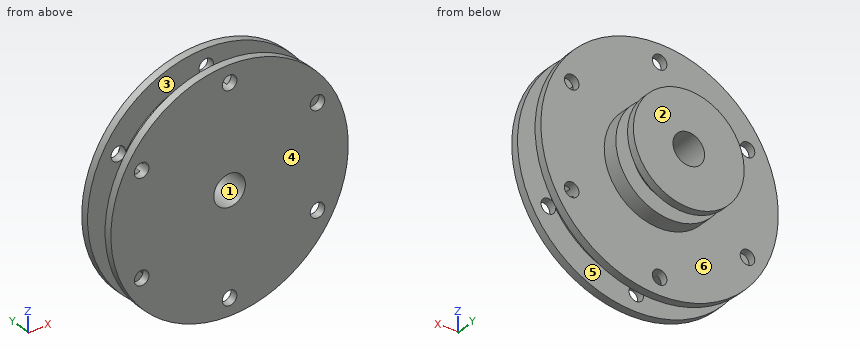
```python
from build123d import *

# Parameters (mm, degrees)
SKETCH1_R               = 15
BOSS_EXTRUDE1_DEPTH     = 5
SKETCH2_W               = 3
SKETCH2_H               = 3
SKETCH3_R               = 7
BOSS_EXTRUDE2_DEPTH     = 5
SKETCH4_W               = 2
SKETCH4_H               = 2
SKETCH5_R               = 2
CUT_EXTRUDE1_DEPTH      = 24.452078799
CUT_EXTRUDE2_DEPTH      = 22.794494718
CUT_EXTRUDE2_DEPTH_BACK = 22.794494718
SKETCH6_R               = 0.920579976


with BuildPart() as part:
    # Sketch1 → Boss-Extrude1 (new body)
    with BuildSketch(Plane(origin=(0, 0, 0), x_dir=(1, 0, 0), z_dir=(0, 1, 0))):
        with Locations(Location((0, 0, 0), (0, 0, 270))):
            Circle(SKETCH1_R)
    extrude(amount=BOSS_EXTRUDE1_DEPTH)

    # Sketch2 → Cut-Revolve1 (revolve, cut)
    with BuildSketch(Plane.XY, mode=Mode.PRIVATE) as cut_revolve1_sk:
        with Locations((13.5, 2.5)):
            Rectangle(SKETCH2_W, SKETCH2_H)
    revolve(cut_revolve1_sk.sketch.rotate(Axis((0, 0, 0), (0, 1, 0)), 90), axis=Axis((0, 0, 0), (0, 1, 0)), mode=Mode.SUBTRACT)

    # Sketch3 → Boss-Extrude2 (add)
    with BuildSketch(Plane(origin=(0, 5, 0), x_dir=(1, 0, 0), z_dir=(0, 1, 0))):
        with Locations(Location((0, 0, 0), (0, 0, 270))):
            Circle(SKETCH3_R)
    extrude(amount=BOSS_EXTRUDE2_DEPTH)

    # Sketch4 → Cut-Revolve2 (revolve, cut)
    with BuildSketch(Plane.XY, mode=Mode.PRIVATE) as cut_revolve2_sk:
        with Locations((6, 8)):
            Rectangle(SKETCH4_W, SKETCH4_H)
    revolve(cut_revolve2_sk.sketch.rotate(Axis((0, 0, 0), (0, 1, 0)), 90), axis=Axis((0, 0, 0), (0, 1, 0)), mode=Mode.SUBTRACT)

    # Sketch5 → Cut-Extrude1 (cut, through all)
    with BuildSketch(Plane(origin=(0, 10, 0), x_dir=(1, 0, 0), z_dir=(0, 1, 0))):
        with Locations(Location((0, 0, 0), (0, 0, 270))):
            Circle(SKETCH5_R)
    extrude(amount=-CUT_EXTRUDE1_DEPTH, mode=Mode.SUBTRACT)

    # Sketch6 → Cut-Extrude2 (cut, two sides: drawn at the far end of the back side and taken through both)
    with BuildSketch(Plane(origin=(0, 5, 0), x_dir=(1, 0, 0), z_dir=(0, 1, 0)).offset(-CUT_EXTRUDE2_DEPTH_BACK)):
        with Locations(Location((0, 12.829886063, 0), (0, 0, 270))):
            Circle(SKETCH6_R)
        with Locations(Location((11.111007258, 6.414943031, 0), (0, 0, 270))):
            Circle(SKETCH6_R)
        with Locations(Location((11.111007258, -6.414943031, 0), (0, 0, 270))):
            Circle(SKETCH6_R)
        with Locations(Location((0, -12.829886063, 0), (0, 0, 270))):
            Circle(SKETCH6_R)
        with Locations(Location((-11.111007258, -6.414943031, 0), (0, 0, 270))):
            Circle(SKETCH6_R)
        with Locations(Location((-11.111007258, 6.414943031, 0), (0, 0, 270))):
            Circle(SKETCH6_R)
    extrude(amount=CUT_EXTRUDE2_DEPTH + CUT_EXTRUDE2_DEPTH_BACK, mode=Mode.SUBTRACT)


solid = part.part
```
Verification items for the finished model (mm, model axes). Face numbers are marked on the shaded views. A direction names the side the tool comes from. Round coordinates to 2 decimals unless told otherwise and drop trailing zeros. Order: outer loops, then holes, each group sorted by start corner. A loop starts at its lowest first (then second) coordinate and runs counter-clockwise, first axis right, second up.
1) Material ranges on line 1 (Z direction, x = 11, y = 4.5); line 2 (Y direction, x = 12.25, z = 1.75); line 3 (Y direction, x = -4.75, z = 1.75), recorded low to high.
Geometry says:
line 1: z = -10.2 to -7.33, -5.5 to 5.5, 7.33 to 10.2
line 2: y = 0 to 1, 4 to 5
line 3: y = 0 to 7, 9 to 10
2) Tool access check on the marked faces 4, 5 and 6. Record the directions out of +Z, -Z, +X, -X, +Y, -Y that give a thin tool (end or side, any length) a straight path to the whole face; none if there is none.
Geometry says:
face 4: +Z, -Z, +X, -X, -Y
face 5: none
face 6: +Y
3) Cross-section at B-B, the plane y = 2.25. Record the cut outline in (x, z), plus the area to 3 significant figures.
Geometry says:
outline: (-10.58, -5.66) arc R0.92 cw to (-10.19, -6.33) arc R12 ccw to (-0.39, -11.99) arc R0.92 cw to (0.39, -11.99) arc R12 ccw to (10.19, -6.33) arc R0.92 cw to (10.58, -5.66) arc R12 ccw to (10.58, 5.66) arc R0.92 cw to (10.19, 6.33) arc R12 ccw to (0.39, 11.99) arc R0.92 cw to (-0.39, 11.99) arc R12 ccw to (-10.19, 6.33) arc R0.92 cw to (-10.58, 5.66) arc R12 ccw to start; hole circle Ø4 at (0, 0)
area: 440 mm2
4) Cross-section at D-D, the plane y = 4.5. Record the cut outline in (x, z), plus the area to 3 significant figures.
Geometry says:
outline: circle Ø30 at (0, 0); hole circle Ø1.84 at (-11.11, -6.41); hole circle Ø1.84 at (-11.11, 6.41); hole circle Ø4 at (0, 0); hole circle Ø1.84 at (0, -12.83); hole circle Ø1.84 at (0, 12.83); hole circle Ø1.84 at (11.11, -6.41); hole circle Ø1.84 at (11.11, 6.41)
area: 678 mm2
5) Draft check along Y on the marked faces 1, 2 and 3. Enter one of: +Y half, -Y half, draft (parallel to the pull), parting line (faces both ways), or undercut.
Geometry says:
face 1: draft
face 2: +Y half
face 3: undercut
6) Cross-section at C-C, the plane x = 5.5. Record the cut outline in (y, z).
Geometry says:
outline: (0, -13.96) - (1, -13.96) - (1, -10.67) - (4, -10.67) - (4, -13.96) - (5, -13.96) - (5, -4.33) - (7, -4.33) - (7, 4.33) - (5, 4.33) - (5, 13.96) - (4, 13.96) - (4, 10.67) - (1, 10.67) - (1, 13.96) - (0, 13.96) - close; (9, -4.33) - (10, -4.33) - (10, 4.33) - (9, 4.33) - close
7) Depth check by flat-ended pin: pin 1 (6 mm diameter, centred on y = 1.5, z = -10.5, fed in from -X); pin 2 (5 mm diameter, centred on y = 5.5, z = 7.5, fed in from +X); pin 3 (4 mm diameter, centred on x = 8, y = 1, fed in from -Z). Enter the tip coordinate at first touch or a pass-through.
Geometry says:
pin 1: stops at x = -12.97
pin 2: stops at x = 14.12
pin 3: stops at z = -13.75
8) Cross-section at A-A, the plane z = 0. Record the cut outline in (x, y), plus the area to 3 significant figures.
Geometry says:
outline: (-15, 0) - (-2, 0) - (-2, 10) - (-7, 10) - (-7, 9) - (-5, 9) - (-5, 7) - (-7, 7) - (-7, 5) - (-15, 5) - (-15, 4) - (-12, 4) - (-12, 1) - (-15, 1) - close; (2, 0) - (15, 0) - (15, 1) - (12, 1) - (12, 4) - (15, 4) - (15, 5) - (7, 5) - (7, 7) - (5, 7) - (5, 9) - (7, 9) - (7, 10) - (2, 10) - close
area: 154 mm2
